```python
from build123d import *

# Parameters (mm, degrees)
SKETCH2_W           = 466
SKETCH2_H           = 466
SKETCH2_W_2         = 450
SKETCH2_H_2         = 450
BOSS_EXTRUDE1_DEPTH = 300
SKETCH4_W           = 8
SKETCH4_H           = 466
BOSS_EXTRUDE2_DEPTH = 450
SKETCH5_W           = 450
SKETCH5_H           = 450
CUT_EXTRUDE1_DEPTH  = 8
SKETCH6_W           = 450
SKETCH6_H           = 450
CUT_EXTRUDE2_DEPTH  = 8


with BuildPart() as part:
    # Sketch2 → Boss-Extrude1 (new, symmetric)
    with BuildSketch(Plane.XY):
        Rectangle(SKETCH2_W, SKETCH2_H)
        Rectangle(SKETCH2_W_2, SKETCH2_H_2, mode=Mode.SUBTRACT)
    extrude(amount=BOSS_EXTRUDE1_DEPTH, both=True)

    # Sketch4 → Boss-Extrude2 (add)
    with BuildSketch(Plane(origin=(-225, 0, 0), x_dir=(0, 0, -1), z_dir=(1, 0, 0))):
        with Locations((296, 0)):
            Rectangle(SKETCH4_W, SKETCH4_H)
    extrude(amount=BOSS_EXTRUDE2_DEPTH)

    # Sketch5 → Cut-Extrude1 (cut)
    with BuildSketch(Plane(origin=(0, 233, 0), x_dir=(1, 0, 0), z_dir=(0, 1, 0))):
        with Locations((0, 67)):
            Rectangle(SKETCH5_W, SKETCH5_H)
    extrude(amount=-CUT_EXTRUDE1_DEPTH, mode=Mode.SUBTRACT)

    # Sketch6 → Cut-Extrude2 (cut)
    with BuildSketch(Plane(origin=(233, 0, 0), x_dir=(0, 0, -1), z_dir=(1, 0, 0))):
        with Locations((67, 0)):
            Rectangle(SKETCH6_W, SKETCH6_H)
    extrude(amount=-CUT_EXTRUDE2_DEPTH, mode=Mode.SUBTRACT)


solid = part.part
```
CAD build for the part. Positions are in the model's coordinates, mm. A direction names the side the tool comes from. Coordinates: 2 decimals unless noted, no trailing zeros. Loops run counter-clockwise (first coordinate to the right, second up) from the corner with the lowest first, then second, coordinate; pieces in that order, holes last. Notation, with made-up numbers: (73, -19) - (99, -19) arc R16 ccw to (99, -14) - close; hole circle Ø3 at (58.5, -3). An arc over 180 degrees is marked (long way). Use CSV: the item, a comma, the result in double quotes. Start each with the question number.
Q1. 3-axis set-ups, long thin cutter, end or side, ignore diameter. For faces 1 (the flat face through (-3, -233, 4)), 2 (the flat face through (-3, 225, 230)): which of +Z, -Z, +X, -X, +Y, -Y reach the whole face in a straight line?
Q2. Probe probe 1 along Y at (x, z) = (-149, 192.5); probe 2 along Z at (x, y) = (8, 90.5). List the from-to ranges inside material, lowest first. Write a range as from..to.
Q3. Two-plate mould, pull along X, no slides. Class faces 3 (the flat face through (1, -225, 8)), 4 (the flat face through (-18, 233, 201)), 5 (the flat face through (233, -18, 201)): +X half, -X half, draft (parallel to the pull), parting line (faces both ways), or undercut.
Q4. Cut at A-A, the plane y = 156. List the corners of the cut face in (x, z).
Q5. Drop flat-ended pins along their axis: P1, Ø6, axis at y = 7.5, z = -85.5, coming from the +X side; P2, Ø2, axis at x = 181, z = -93.5, coming from the +Y side; P3, Ø5, axis at x = -183.5, y = -127.5, coming from the +Z side. Give the stop position or say it passes through.
Q6. Cut at C-C, the plane z = 226. List the corners of the cut face in (x, y).
Q7. Cut at B-B, the plane z = 17.5. List the corners of the cut face in (x, y).
Here are the results:
1,face 1,"+Z, -Z, +X, -X, -Y"
1,face 2,"+Z"
2,probe 1,"-233..-225, 225..233"
2,probe 2,"-300..-292"
3,face 3,"undercut"
3,face 4,"draft"
3,face 5,"+X half"
4,outline,"(-233, -300) - (233, -300) - (233, -292) - (-225, -292) - (-225, 300) - (-233, 300) - close; (225, 158) - (233, 158) - (233, 300) - (225, 300) - close"
5,P1,"x = -225"
5,P2,"y = -225"
5,P3,"z = -292"
6,outline,"(-233, -233) - (233, -233) - (233, 233) - (-233, 233) - close; hole (-225, -225) - (225, -225) - (225, 225) - (-225, 225) - close"
7,outline,"(-233, -233) - (233, -233) - (233, -225) - (-225, -225) - (-225, 233) - (-233, 233) - close; (225, 225) - (233, 225) - (233, 233) - (225, 233) - close"
